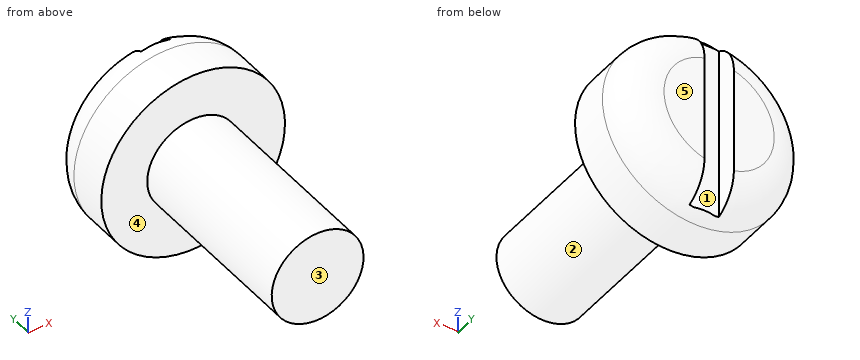
from build123d import *

# Parameters (mm, degrees)
HEAD_EDGE_FILLET_R1_R            = 1
SCREWDRIVER_SLOT_SKETCH_W        = 0.8
SCREWDRIVER_SLOT_SKETCH_H        = 4.8
SCREWDRIVER_SLOT_0_8_X_0_6_DEPTH = 0.6


with BuildPart() as part:
    # Bolt Profile Sketch → Bolt Body Ø2.5 Shank Ø5 Head (revolve)
    with BuildSketch(Plane.XY, mode=Mode.PRIVATE) as bolt_body_2_5_shank_5_head_sk:
        Polygon((0, -5), (1.25, -5), (1.25, 0), (2.5, 0), (2.5, 2.1), (0, 2.1), align=None)
    revolve(bolt_body_2_5_shank_5_head_sk.sketch.rotate(Axis((0, 4.110962567, 0), (0, -1, 0)), 90), axis=Axis((0, 4.110962567, 0), (0, -1, 0)))

    # Head Edge Fillet R1
    head_edge_fillet_r1_edges = [part.edges().sort_by_distance(p)[0] for p in [
        (0, 2.1, -2.5),
    ]]
    fillet(head_edge_fillet_r1_edges, radius=HEAD_EDGE_FILLET_R1_R)

    # Screwdriver Slot Sketch → Screwdriver Slot 0.8 x 0.6 (cut)
    with BuildSketch(Plane(origin=(0, 2.1, 0), x_dir=(1, 0, 0), z_dir=(0, 1, 0))):
        Rectangle(SCREWDRIVER_SLOT_SKETCH_W, SCREWDRIVER_SLOT_SKETCH_H)
    extrude(amount=-SCREWDRIVER_SLOT_0_8_X_0_6_DEPTH, mode=Mode.SUBTRACT)


solid = part.part
For this review, take the finished solid that the model builds, in its own axes (mm). Face numbers are marked on the shaded views. A direction names the side the tool comes from. Round coordinates to 2 decimals unless told otherwise and drop trailing zeros. Order: outer loops, then holes, each group sorted by start corner. A loop starts at its lowest first (then second) coordinate and runs counter-clockwise, first axis right, second up. Notation, with made-up numbers: M -16.5,-1 L 7.5,-1 A35 cw 7.5,31 Z; hole C -35,55.5 d2. An arc over 180 degrees is marked long. Use a Markdown table: item, result. Add a question column.
Item 1: Mouldability with a two-part tool opening along Z and no side actions: class the marked faces 1, 2 and 3 as released by +Z, released by -Z, zero draft, split by the parting line, or undercut.
Item 2: Insertion check: pin 1 (0.6 mm diameter, centred on x = 0, z = 0.5, fed in from +Y); pin 2 (0.7 mm diameter, centred on y = 2, z = 0.5, fed in from +X); pin 3 (3 mm diameter, centred on x = -0.5, y = -3, fed in from +Z). Each pin has a flat end and moves straight along its axis. Give the tip position at first contact, or say it passes through.
Item 3: To check wall thickness, follow line 1 along Y through (x, z) = (-0.45, 1.2); line 2 along Y through (x, z) = (-0.1, -1.3); line 3 along X through (y, z) = (-4, 0.25). State the ranges of each line that lie inside material, in increasing order.
Item 4: Add section A-A, the plane z = 0. Give the boundary of the cut face in (x, y).
Item 5: Tool access review of the marked faces 4 and 5: name each direction out of +Z, -Z, +X, -X, +Y, -Y from which nothing blocks a thin tool from reaching the whole face with its end or side.
Item 6: Add section D-D, the plane y = 0.5. Give the boundary of the cut face in (x, z), then the cut area to 3 significant figures.
Item 7: Add section C-C, the plane y = -2. Give the boundary of the cut face in (x, z).
Geometry results:
| question | item | result |
|---|---|---|
| 1 | face 1 | undercut |
| 1 | face 2 | split by the parting line |
| 1 | face 3 | zero draft |
| 2 | pin 1 | stops at y = 1.5 |
| 2 | pin 2 | stops at x = 2.29 |
| 2 | pin 3 | stops at z = 1.25 |
| 3 | line 1 | y = 0 to 2.1 |
| 3 | line 2 | y = 0 to 1.5 |
| 3 | line 3 | x = -1.22 to 1.22 |
| 4 | outline | M -2.5,0 L -1.25,0 L -1.25,-5 L 1.25,-5 L 1.25,0 L 2.5,0 L 2.5,1.1 A1 ccw 1.5,2.1 L 0.4,2.1 L 0.4,1.5 L -0.4,1.5 L -0.4,2.1 L -1.5,2.1 A1 ccw -2.5,1.1 Z |
| 5 | face 4 | -Y |
| 5 | face 5 | +Z, -Z, +X, -X, +Y |
| 6 | outline | C 0,0 d5 |
| 6 | area | 19.6 mm² |
| 7 | outline | C 0,0 d2.5 |
